The model under review builds one solid part; all positions refer to its coordinate system, in mm. A direction names the side the tool comes from. Coordinates: 2 decimals unless noted, no trailing zeros. Order: outer loops, then holes, each group sorted by start corner. A loop starts at its lowest first (then second) coordinate and runs counter-clockwise, first axis right, second up. Notation, with made-up numbers: M -4,19 L 30,19 A26 cw 30,35 Z; hole C 33.25,61.25 d9. An arc over 180 degrees is marked long. Write each question's results on one line, items separated by ' | '.
from build123d import *

# Parameters (mm, degrees)
SKETCH1_W           = 200
SKETCH1_H           = 5
BOSS_EXTRUDE1_DEPTH = 500
SKETCH2_W           = 75
SKETCH2_H           = 10
BOSS_EXTRUDE2_DEPTH = 500


with BuildPart() as part:
    # Sketch1 → Boss-Extrude1 (new body)
    with BuildSketch(Plane.XY):
        Rectangle(SKETCH1_W, SKETCH1_H)
    extrude(amount=BOSS_EXTRUDE1_DEPTH)

    # Sketch2 → Boss-Extrude2 (add)
    with BuildSketch(Plane.XY.offset(500)):
        Rectangle(SKETCH2_W, SKETCH2_H)
    extrude(amount=-BOSS_EXTRUDE2_DEPTH)


solid = part.part
1) For faces 1 (the flat face through (-1, 0, 0)), 2 (the flat face through (-69, 2.5, 246)), 3 (the flat face through (-69, -2.5, 246)), 4 (the flat face through (68, 2.5, 246)), 5 (the flat face through (68, -2.5, 246)), list the 3-axis set-ups (+Z, -Z, +X, -X, +Y, -Y) from which the entire face can be reached by the end or side of a thin tool; tool diameter is ignored.
Solutions:
face 1: -Z, +X, -X, +Y, -Y | face 2: +Z, -Z, -X, +Y | face 3: +Z, -Z, -X, -Y | face 4: +Z, -Z, +X, +Y | face 5: +Z, -Z, +X, -Y
2) Take a section at A-A on z = 125.5. State the section outline as (x, y) points, plus the area to 4 significant figures.
Solutions:
outline: M -100,-2.5 L -37.5,-2.5 L -37.5,-5 L 37.5,-5 L 37.5,-2.5 L 100,-2.5 L 100,2.5 L 37.5,2.5 L 37.5,5 L -37.5,5 L -37.5,2.5 L -100,2.5 Z | area: 1,375 mm2
3) To check wall thickness, follow line 1 along Y through (x, z) = (52, 109); line 2 along X through (y, z) = (-2.75, 340). State the ranges of each line that lie inside material, in increasing order.
Solutions:
line 1: -2.5 to 2.5 | line 2: -37.5 to 37.5
4) For pin 1 (1.2 mm diameter, centred on y = -3, z = 240, fed in from +X); pin 2 (19 mm diameter, centred on x = -76.5, z = 304.5, fed in from +Y); pin 3 (1.2 mm diameter, centred on y = 4.5, z = 199, fed in from -X); pin 4 (1.5 mm diameter, centred on x = -44.5, z = 60.5, fed in from -Y), all flat-tipped, find the tip position at first contact; note any pin that passes through.
Solutions:
pin 1: x = 100 | pin 2: y = 2.5 | pin 3: x = -37.5 | pin 4: y = -2.5
5) Take a section at B-B on x = 87. State the section outline as (y, z) points.
Solutions:
outline: M -2.5,0 L 2.5,0 L 2.5,500 L -2.5,500 Z
